Can you work these out from the model? Positions are in its coordinate system, mm. Face numbers are marked on the shaded views. A direction names the side the tool comes from. Coordinates: 2 decimals unless noted, no trailing zeros. Loops run counter-clockwise (first coordinate to the right, second up) from the corner with the lowest first, then second, coordinate; pieces in that order, holes last. Notation, with made-up numbers: (80, 0.5) - (124, 0.5) arc R23 ccw to (124, 39.5) - close; hole circle Ø10 at (54.5, -31.75). An arc over 180 degrees is marked (long way). Put each result on its own line as item: value. Start each with the question number.
from build123d import *

# Parameters (mm, degrees)
SKETCH1_R           = 11
BOSS_EXTRUDE1_DEPTH = 4.5
SKETCH2_R           = 9
BOSS_EXTRUDE2_DEPTH = 30
SKETCH3_R           = 10
BOSS_EXTRUDE3_DEPTH = 51
BOSS_EXTRUDE4_START = 10
SKETCH4_R           = 9
BOSS_EXTRUDE4_DEPTH = 10
CUT_EXTRUDE1_DEPTH  = 15
BOSS_EXTRUDE5_DEPTH = 6
CUT_EXTRUDE2_DEPTH  = 19
BOSS_EXTRUDE6_DEPTH = 6
CHAMFER1_SIZE       = 0.5
SKETCH9_R           = 8
BOSS_EXTRUDE7_DEPTH = 35
CHAMFER2_SIZE       = 0.5
SKETCH10_R          = 2.5
CUT_EXTRUDE3_DEPTH  = 15


with BuildPart() as part:
    # Sketch1 → Boss-Extrude1 (new, symmetric)
    with BuildSketch(Plane.XY):
        Circle(SKETCH1_R)
    extrude(amount=BOSS_EXTRUDE1_DEPTH, both=True)

    # Sketch2 → Boss-Extrude2 (add)
    with BuildSketch(Plane(origin=(0, 0, -4.5), x_dir=(-1, 0, 0), z_dir=(0, 0, -1))):
        with Locations(Location((0, 0, 0), (0, 0, 180))):
            Circle(SKETCH2_R)
    extrude(amount=BOSS_EXTRUDE2_DEPTH)

    # Sketch3 → Boss-Extrude3 (add)
    with BuildSketch(Plane.XY.offset(4.5)):
        Circle(SKETCH3_R)
    extrude(amount=BOSS_EXTRUDE3_DEPTH)

    # Sketch4 → Boss-Extrude4 (add)
    with BuildSketch(Plane.XY.offset(55.5).offset(BOSS_EXTRUDE4_START)):
        Circle(SKETCH4_R)
    extrude(amount=-BOSS_EXTRUDE4_DEPTH)

    # Sketch5 → Cut-Extrude1 (cut)
    with BuildSketch(Plane(origin=(0, 0, 0), x_dir=(1, 0, 0), z_dir=(0, 1, 0))):
        with BuildLine():
            Line((-3, -65.5), (-3, -59.5))
            ThreePointArc((-3, -59.5), (0, -56.5), (3, -59.5))
            Line((3, -59.5), (3, -65.5))
            ThreePointArc((3, -65.5), (0, -68.5), (-3, -65.5))
        make_face()
    extrude(amount=-CUT_EXTRUDE1_DEPTH, mode=Mode.SUBTRACT)

    # Sketch6 → Boss-Extrude5 (add)
    with BuildSketch(Plane.XZ):
        with BuildLine():
            Line((3, 65.5), (-3, 65.5))
            Line((-3, 65.5), (-3, 59.5))
            ThreePointArc((-3, 59.5), (0, 56.5), (3, 59.5))
            Line((3, 59.5), (3, 65.5))
        make_face()
    extrude(amount=BOSS_EXTRUDE5_DEPTH)

    # Sketch7 → Cut-Extrude2 (cut)
    with BuildSketch(Plane(origin=(0, 0, 0), x_dir=(1, 0, 0), z_dir=(0, 1, 0))):
        with BuildLine():
            Line((3, 10.5), (3, 8.5))
            ThreePointArc((3, 8.5), (0, 5.5), (-3, 8.5))
            Line((-3, 8.5), (-3, 10.5))
            ThreePointArc((-3, 10.5), (0, 13.5), (3, 10.5))
        make_face()
    extrude(amount=-CUT_EXTRUDE2_DEPTH, mode=Mode.SUBTRACT)

    # Sketch8 → Boss-Extrude6 (add)
    with BuildSketch(Plane.XZ):
        with BuildLine():
            Line((3, -10.5), (3, -8.5))
            ThreePointArc((3, -8.5), (0, -5.5), (-3, -8.5))
            Line((-3, -8.5), (-3, -10.5))
            ThreePointArc((-3, -10.5), (0, -13.5), (3, -10.5))
        make_face()
    extrude(amount=BOSS_EXTRUDE6_DEPTH)

    # Chamfer1
    chamfer1_edges = [part.edges().sort_by_distance(p)[0] for p in [
        (-10, 0, 55.5),
        (-5.196152423, 7.348469228, 65.5),
        (-11, 0, -4.5),
        (-11, 0, 4.5),
        (-9, 0, -34.5),
    ]]
    chamfer(chamfer1_edges, length=CHAMFER1_SIZE)

    # Sketch9 → Boss-Extrude7 (add)
    with BuildSketch(Plane(origin=(0, 0, -34.5), x_dir=(-1, 0, 0), z_dir=(0, 0, -1))):
        Circle(SKETCH9_R)
    extrude(amount=BOSS_EXTRUDE7_DEPTH)

    # Chamfer2
    chamfer2_edges = [part.edges().sort_by_distance(p)[0] for p in [
        (8, 0, -69.5),
    ]]
    chamfer(chamfer2_edges, length=CHAMFER2_SIZE)

    # Sketch10 → Cut-Extrude3 (cut, symmetric)
    with BuildSketch(Plane(origin=(0, 0, 0), x_dir=(1, 0, 0), z_dir=(0, 1, 0))):
        with Locations(Location((0, 49.5, 0), (0, 0, 270))):
            Circle(SKETCH10_R)
    extrude(amount=CUT_EXTRUDE3_DEPTH, both=True, mode=Mode.SUBTRACT)


solid = part.part
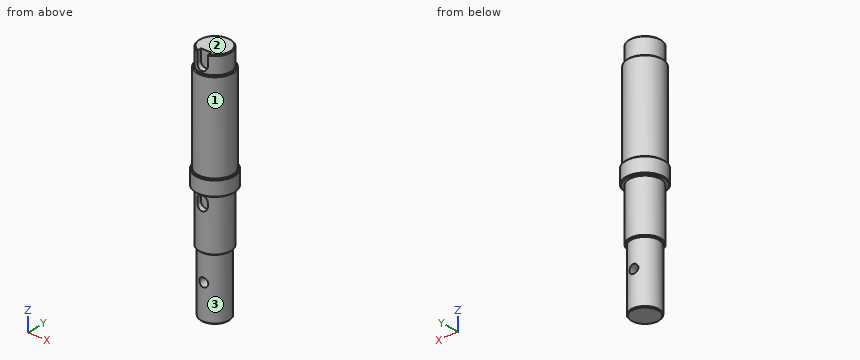
Q1. I want a section at B-B on z = -49.5. List the corners of the cut face in (x, y) for me, and give its area (3 significant figures).
Q2. Please list where these lines run through material, in increasing order: line 1 along Z through (x, y) = (0, 3.5); line 2 along X through (y, z) = (0.5, -49.5); line 3 along Y through (x, z) = (-6, 36). Write a range as [from, to].
Q3. Will these pins go through, and if not, where does the flat tip stop? pin 1 (2 mm diameter, centred on y = -7.5, z = -9.5, fed in from -X); pin 2 (1.2 mm diameter, centred on y = -7, z = 63, fed in from +X); pin 3 (2 mm diameter, centred on x = 1.5, z = 14.5, fed in from -Y).
Q4. On a 3-axis mill with a long thin cutter (end or side, diameter ignored), from which of +Z, -Z, +X, -X, +Y, -Y can I reach the whole of each face in a straight line? I mean the marked faces 1, 2 and 3. Say none if no direction works.
Q5. I want a section at A-A on z = -32. List the corners of the cut face in (x, y) for me.
Calculated:
1. outline: (-2.5, -7.6) - (-2.5, 7.6) arc R8 ccw to start; (2.5, -7.6) arc R8 ccw to (2.5, 7.6) - close
1. area: 122 mm2
2. line 1: [-69.5, -52], [-47, 65.5]
2. line 2: [-7.98, -2.5], [2.5, 7.98]
2. line 3: [-8, 8]
3. pin 1: x = -6.22
3. pin 2: x = 6.33
3. pin 3: y = -9.99
4. face 1: +Z
4. face 2: +Z, +X, -X, +Y, -Y
4. face 3: -Z
5. outline: circle Ø18 at (0, 0)
